from build123d import *

# Parameters (mm, degrees)
EXTRUDE_1_DEPTH     = 32
FILLET_1_R          = 0.5
FILLET_2_R          = 2
FILLET_3_R          = 5
CUT_EXTRUDE_1_REACH = 59
SKETCH_2_R          = 1.75
CUT_EXTRUDE_2_REACH = 57.958


with BuildPart() as part:
    # 草图1 → 拉伸-薄壁1 (new body)
    with BuildSketch(Plane.XY):
        Polygon((25, 0), (0, 0), (0, 40), (1.5, 40), (1.5, 1.5), (25, 1.5), align=None)
    extrude(amount=EXTRUDE_1_DEPTH)

    # 圆角1
    fillet_1_edges = [part.edges().sort_by_distance(p)[0] for p in [
        (1.5, 1.5, 16),
    ]]
    fillet(fillet_1_edges, radius=FILLET_1_R)

    # 圆角2
    fillet_2_edges = [part.edges().sort_by_distance(p)[0] for p in [
        (0, 0, 16),
    ]]
    fillet(fillet_2_edges, radius=FILLET_2_R)

    # 圆角3
    fillet_3_edges = [part.edges().sort_by_distance(p)[0] for p in [
        (0.75, 40, 32),
        (0.75, 40, 0),
        (25, 0.75, 0),
        (25, 0.75, 32),
    ]]
    fillet(fillet_3_edges, radius=FILLET_3_R)

    # 草图2 → 切除-拉伸1 (cut, up to next)
    with BuildSketch(Plane.ZY, mode=Mode.PRIVATE) as cut_extrude_1_sk1:
        with Locations((3.3, 20)):
            Circle(SKETCH_2_R)
    cut_extrude_1_tool1 = extrude(cut_extrude_1_sk1.sketch, amount=-CUT_EXTRUDE_1_REACH, mode=Mode.PRIVATE) & part.part
    # 草图2 → 切除-拉伸1 (cut, up to next)
    with BuildSketch(Plane.ZY, mode=Mode.PRIVATE) as cut_extrude_1_sk2:
        with Locations((28.7, 20)):
            Circle(SKETCH_2_R)
    cut_extrude_1_tool2 = extrude(cut_extrude_1_sk2.sketch, amount=-CUT_EXTRUDE_1_REACH, mode=Mode.PRIVATE) & part.part
    add(cut_extrude_1_tool1.solids().sort_by_distance((0, 20, 3.3))[0], mode=Mode.SUBTRACT)
    add(cut_extrude_1_tool2.solids().sort_by_distance((0, 20, 28.7))[0], mode=Mode.SUBTRACT)

    # 草图3 → 切除-拉伸2 (cut, up to next)
    with BuildSketch(Plane(origin=(0, 1.5, 0), x_dir=(1, 0, 0), z_dir=(0, 1, 0)), mode=Mode.PRIVATE) as cut_extrude_2_sk1:
        with BuildLine():
            Line((5, -3.75), (20, -3.75))
            ThreePointArc((20, -3.75), (22.25, -6), (20, -8.25))
            Line((20, -8.25), (5, -8.25))
            ThreePointArc((5, -8.25), (2.75, -6), (5, -3.75))
        make_face()
    cut_extrude_2_tool1 = extrude(cut_extrude_2_sk1.sketch, amount=-CUT_EXTRUDE_2_REACH, mode=Mode.PRIVATE) & part.part
    # 草图3 → 切除-拉伸2 (cut, up to next)
    with BuildSketch(Plane(origin=(0, 1.5, 0), x_dir=(1, 0, 0), z_dir=(0, 1, 0)), mode=Mode.PRIVATE) as cut_extrude_2_sk2:
        with BuildLine():
            Line((5, -23.75), (20, -23.75))
            ThreePointArc((20, -23.75), (22.25, -26), (20, -28.25))
            Line((20, -28.25), (5, -28.25))
            ThreePointArc((5, -28.25), (2.75, -26), (5, -23.75))
        make_face()
    cut_extrude_2_tool2 = extrude(cut_extrude_2_sk2.sketch, amount=-CUT_EXTRUDE_2_REACH, mode=Mode.PRIVATE) & part.part
    add(cut_extrude_2_tool1.solids().sort_by_distance((12.5, 1.5, 6))[0], mode=Mode.SUBTRACT)
    add(cut_extrude_2_tool2.solids().sort_by_distance((12.5, 1.5, 26))[0], mode=Mode.SUBTRACT)


solid = part.part
Could you check a few things on this model? Use its own coordinates, in mm. A direction names the side the tool comes from. Give positions to 0.01 mm unless a question says otherwise; leave off trailing zeros. Loops run counter-clockwise (first coordinate to the right, second up) from the corner with the lowest first, then second, coordinate; pieces in that order, holes last. Notation, with made-up numbers: (11.25, 63) -> (23.25, 63) arc R26 cw to (23.25, 81) -> close; hole circle Ø2 at (30.25, 73.5). An arc over 180 degrees is marked (long way). Answer as CSV lines item,"result". Start each with the question number.
(1) If we section it at B-B on x = 10: Write out the boundary of the cut face in (y, z).
(2) If we section it at D-D on z = 12.5: Write out the boundary of the cut face in (x, y), then the cut area to 3 significant figures.
(3) Which directions (+Z, -Z, +X, -X, +Y, -Y) give clear straight access to the entire face, cutting with the end or side of a thin tool? Please do faces 4 (the flat face through (1.5, 21, 16)), 5 (the flat face through (14, 0, 16)), 6 (the flat face through (12, 1, 23.75)).
(4) If we section it at C-C on y = 19: Write out the boundary of the cut face in (x, z).
(5) I need wall thicknesses on probe 1 along X at (y, z) = (10.5, 2.5); probe 2 along Y at (x, z) = (0.4, 3.3). Which ranges of each line are inside material? Lowest first, please.
(6) If we section it at A-A on z = 26: Write out the boundary of the cut face in (x, y).
(7) We'd pull the mould along X, two halves only. Please class faces 1 (the flat face through (25, 1, 16)), 2 (the cylindrical face through (0.74, 21.735, 3.072)), 3 (the cylindrical face through (2.75, 0.76, 6.05)): released by +X, released by -X, zero draft, split by the parting line, or undercut.
(8) I'm going to push flat-ended pins straight in: pin 1 Ø12 at (x, z) = (20.5, 12) entering from -Y; pin 2 Ø6 at (y, z) = (34, 27.5) entering from +X; pin 3 Ø3 at (y, z) = (20, 3.3) entering from +X; pin 4 Ø4 at (x, z) = (11.5, 13.5) entering from +Y. Where does each tip first touch, or does it pass through?
Computed:
1,outline,"(0, 0) -> (1.5, 0) -> (1.5, 3.75) -> (0, 3.75) -> close; (0, 8.25) -> (1.5, 8.25) -> (1.5, 23.75) -> (0, 23.75) -> close; (0, 28.25) -> (1.5, 28.25) -> (1.5, 32) -> (0, 32) -> close"
2,outline,"(0, 2) arc R2 ccw to (2, 0) -> (25, 0) -> (25, 1.5) -> (2, 1.5) arc R0.5 cw to (1.5, 2) -> (1.5, 40) -> (0, 40) -> close"
2,area,"94.4 mm2"
3,face 4,"+Z, -Z, +X, +Y"
3,face 5,"+Z, -Z, +X, -X, -Y"
3,face 6,"+Y, -Y"
4,outline,"(0, 0) -> (1.5, 0) -> (1.5, 1.86) -> (0, 1.86) -> close; (0, 4.74) -> (1.5, 4.74) -> (1.5, 27.26) -> (0, 27.26) -> close; (0, 30.14) -> (1.5, 30.14) -> (1.5, 32) -> (0, 32) -> close"
5,probe 1,"x = 0 to 1.5"
5,probe 2,"y = 0.8 to 18.25, 21.75 to 39.7"
6,outline,"(0, 2) arc R2 ccw to (2, 0) -> (2.75, 0) -> (2.75, 1.5) -> (2, 1.5) arc R0.5 cw to (1.5, 2) -> (1.5, 40) -> (0, 40) -> close; (22.25, 0) -> (25, 0) -> (25, 1.5) -> (22.25, 1.5) -> close"
7,face 1,"released by +X"
7,face 2,"zero draft"
7,face 3,"undercut"
8,pin 1,"stops at y = 0"
8,pin 2,"stops at x = 1.5"
8,pin 3,"passes through"
8,pin 4,"stops at y = 1.5"
